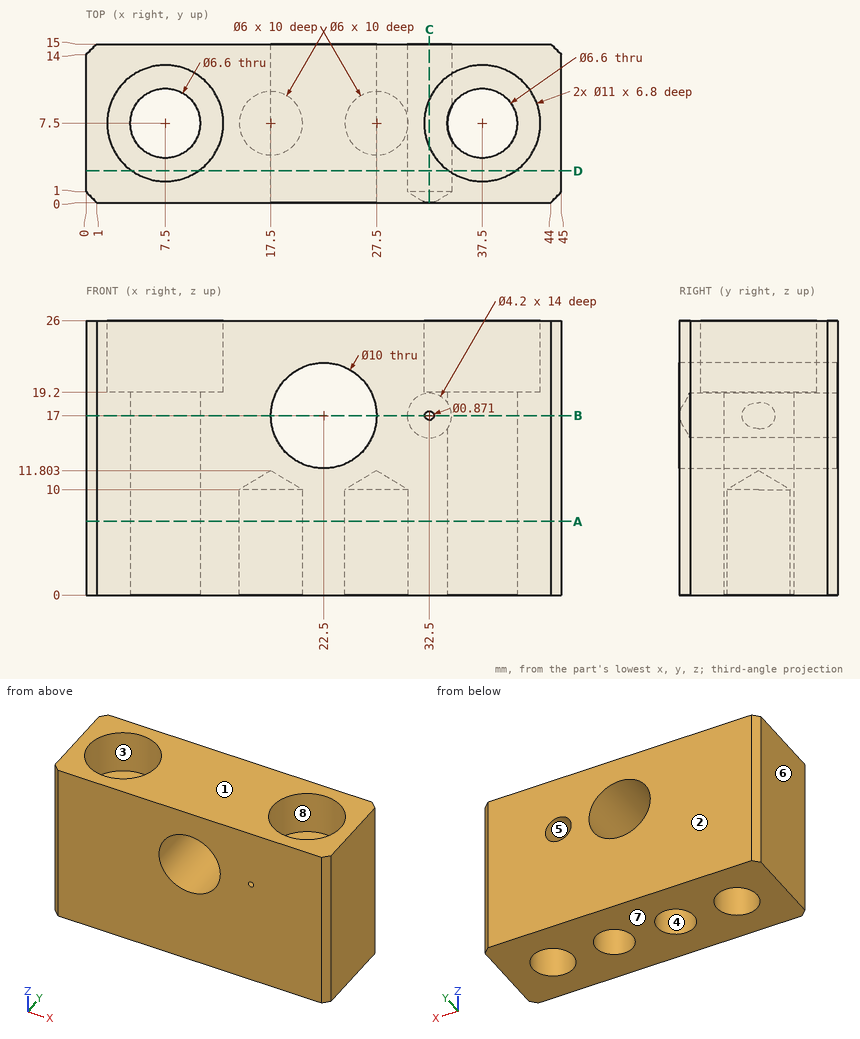
Can you work these out from the drawing? Everything is in mm from the part's minimum corner. A direction names the side the tool comes from. Round coordinates to 2 decimals unless told otherwise and drop trailing zeros. Order: outer loops, then holes, each group sorted by start corner. A loop starts at its lowest first (then second) coordinate and runs counter-clockwise, first axis right, second up.
(1) If we section it at D-D (y = 3): Please give me the cut outline in (x, z).
Results are:
outline: (0, 0) - (45, 0) - (45, 26) - (40.66, 26) - (40.66, 19.2) - (34.34, 19.2) - (34.34, 26) - (10.66, 26) - (10.66, 19.2) - (4.34, 19.2) - (4.34, 26) - (0, 26) - close; hole circle Ø10 at (22.5, 17); hole circle Ø4.2 at (32.5, 17)
(2) I'm going to push flat-ended pins straight in: pin 1 (5.5 mm diameter, centred on x = 35.5, y = 9, fed in from +Z); pin 2 (8 mm diameter, centred on x = 22.5, z = 17, fed in from -Y); pin 3 (5 mm diameter, centred on x = 17.5, y = 7.5, fed in from -Z). Where does each tip first touch, or does it pass through?
Results are:
pin 1: stops at z = 19.2
pin 2: passes through
pin 3: stops at z = 10.3
(3) If we section it at A-A (z = 7): Please give me the cut outline in (x, y), plus the area to 3 significant figures.
Results are:
outline: (0, 1) - (1, 0) - (44, 0) - (45, 1) - (45, 14) - (44, 15) - (1, 15) - (0, 14) - close; hole circle Ø6.6 at (7.5, 7.5); hole circle Ø6 at (17.5, 7.5); hole circle Ø6 at (27.5, 7.5); hole circle Ø6.6 at (37.5, 7.5)
area: 548 mm2
(4) We'd pull the mould along Y, two halves only. Please class the marked faces 1, 2 and 3: +Y half, -Y half, draft (parallel to the pull), parting line (faces both ways), or undercut.
Results are:
face 1: draft
face 2: +Y half
face 3: undercut
(5) If we section it at B-B (z = 17): Please give me the cut outline in (x, y) (1 decimal), plus the area to 3 significant figures.
Results are:
outline: (0, 1) - (1, 0) - (17.5, 0) - (17.5, 15) - (1, 15) - (0, 14) - close; (27.5, 0) - (32.1, 0) - (30.4, 1) - (30.4, 15) - (27.5, 15) - close; (32.9, 0) - (44, 0) - (45, 1) - (45, 14) - (44, 15) - (34.6, 15) - (34.6, 9.1) arc R3.3 cw (long way) to (34.6, 5.9) - (34.6, 1) - close; hole circle Ø6.6 at (7.5, 7.5)
area: 394 mm2
(6) On a 3-axis mill with a long thin cutter (end or side, diameter ignored), from which of +Z, -Z, +X, -X, +Y, -Y can I reach the whole of each face in a straight line? I mean the marked faces 4, 5, 6, 7 and 8. Say none if no direction works.
Results are:
face 4: -Z
face 5: +Y
face 6: +Z, -Z, -X, +Y, -Y
face 7: -Z, +X, -X, +Y, -Y
face 8: +Z
(7) If we section it at C-C (x = 32.5): Please give me the cut outline in (y, z) (1 decimal).
Results are:
outline: (0, 0) - (15, 0) - (15, 14.9) - (1, 14.9) - (0, 16.6) - close; (0, 17.4) - (1, 19.1) - (15, 19.1) - (15, 26) - (9.8, 26) - (9.8, 19.2) - (5.2, 19.2) - (5.2, 26) - (0, 26) - close
(8) If I drill on L1, parallel to X at y = 7.75, z = 23.5 (1 decimal); L2, parallel to Y at x = 37.5, z = 22; L3, parallel to Y at x = 7.5, z = 7.75, over which ranges is the centre line in solid material (lowest first)?
Results are:
L1: x = 0 to 2, 13 to 32, 43 to 45
L2: y = 0 to 2, 13 to 15
L3: y = 0 to 4.2, 10.8 to 15
